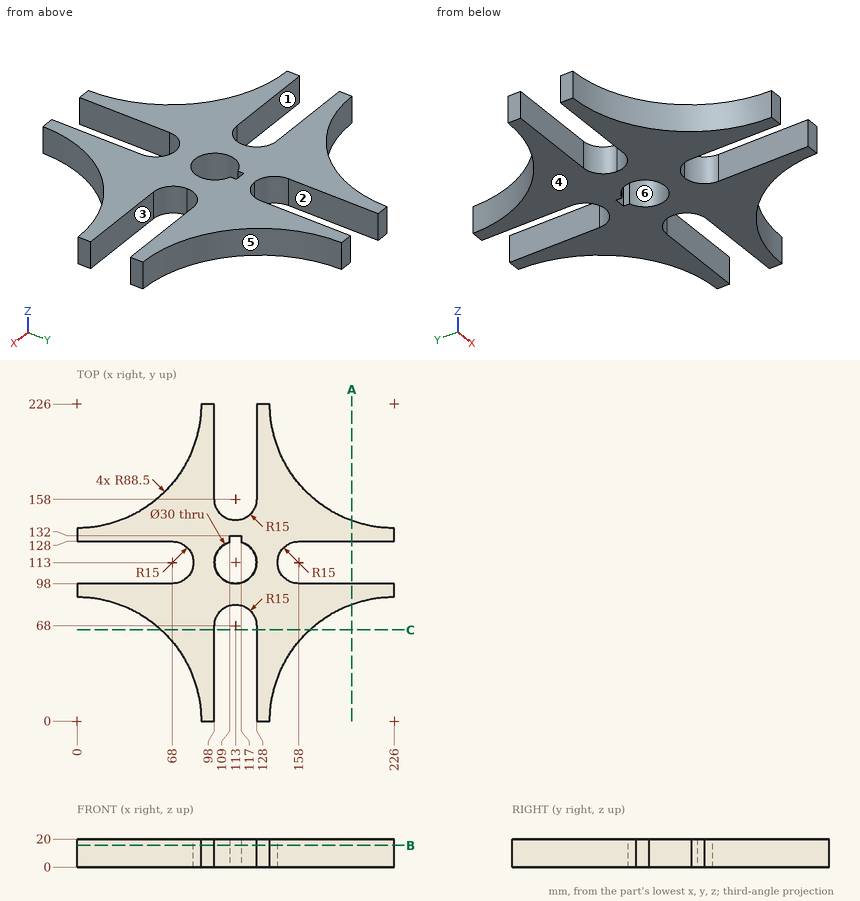
The drawing under review shows one solid part. Ordinate dimensions are in mm from its lowest x, y, z. A direction names the side the tool comes from. Give positions to 0.01 mm unless a question says otherwise; leave off trailing zeros. Loops run counter-clockwise (first coordinate to the right, second up) from the corner with the lowest first, then second, coordinate; pieces in that order, holes last. Notation, with made-up numbers: M -31.5,0.25 L -9.5,0.25 A32 cw -9.5,27.25 Z; hole C 23,27.5 d8. An arc over 180 degrees is marked long. One line per item, written item: value. Start each with the question number.
Q1. For L1, parallel to Y at x = 113, z = 9.75; L2, parallel to X at y = 113, z = 10.25; L3, parallel to Y at x = 55, z = 3, list the stretches that pass through material, from the lowest coordinate up.
Q2. Add section A-A (x = 196). Give the boundary of the cut face in (y, z).
Q3. Add section C-C (y = 65). Give the boundary of the cut face in (x, z), and give its area (3 significant figures).
Q4. Machinability: for the marked faces 1, 2 and 3, which of the approach directions +Z, -Z, +X, -X, +Y, -Y give a long, thin tool a straight path to every point of the face, cutting with its end or side? Answer none if there is none.
Q5. Draft analysis for pull direction Y (two halves, no side actions). For the marked faces 4, 5 and 6, state which applies: released by +Y, released by -Y, zero draft, split by the parting line, or undercut.
Q6. Clearance check with flat-ended pins moving along their axes: pin 1 Ø6 at (y, z) = (183, 7.5) entering from +X; pin 2 Ø6 at (x, z) = (186.5, 12) entering from +Y; pin 3 Ø10 at (x, z) = (63.5, 11.5) entering from +Y; pin 4 Ø5 at (x, y) = (101, 55.5) entering from -Z. State where each tip first meets the part, or that it passes through.
Q7. Add section B-B (z = 15.5). Give the boundary of the cut face in (x, y), and give its area (3 significant figures).
Reply:
1. L1: 83 to 98, 132 to 143
1. L2: 83 to 98, 128 to 143
1. L3: 69.33 to 98, 128 to 156.67
2. outline: M 83.26,0 L 98,0 L 98,20 L 83.26,20 Z; M 128,0 L 142.74,0 L 142.74,20 L 128,20 Z
3. outline: M 60.06,0 L 98,0 L 98,20 L 60.06,20 Z; M 128,0 L 165.94,0 L 165.94,20 L 128,20 Z
3. area: 1,520 mm²
4. face 1: +Z, -Z, -X
4. face 2: +Z, -Z, +Y
4. face 3: +Z, -Z, +X
5. face 4: zero draft
5. face 5: released by +Y
5. face 6: undercut
6. pin 1: x = 150.39
6. pin 2: y = 148.37
6. pin 3: y = 169.96
6. pin 4: through
7. outline: M 0,88.5 A88.5 cw 88.5,0 L 98,0 L 98,68 A15 cw 128,68 L 128,0 L 137.5,0 A88.5 cw 226,88.5 L 226,98 L 158,98 A15 cw 158,128 L 226,128 L 226,137.5 A88.5 cw 137.5,226 L 128,226 L 128,158 A15 cw 98,158 L 98,226 L 88.5,226 A88.5 cw 0,137.5 L 0,128 L 68,128 A15 cw 68,98 L 0,98 Z; hole M 109,127.46 A15 ccw long 117,127.46 L 117,132 L 109,132 Z
7. area: 16,200 mm²
